Part print with two shaded views. Sizes in mm from the minimum x, y, z corner. A direction names the side the tool comes from. Round coordinates to 2 decimals unless told otherwise and drop trailing zeros. Order: outer loops, then holes, each group sorted by start corner. A loop starts at its lowest first (then second) coordinate and runs counter-clockwise, first axis right, second up. Notation, with made-up numbers: M 65,-23.75 L 122,-23.75 A12 cw 122,-12.75 Z; hole C 12,65 d4. An arc over 180 degrees is marked long. Return JSON: item names as keys, results as strings. Group by question number.
Item 1: Slice it at D-D on x = 10.5. Write the cut outline in (y, z).
Item 2: Which spindle directions (+Z, -Z, +X, -X, +Y, -Y) get a long thin tool onto all of the face, cutting with end or side? Do the marked faces 4, 5 and 6. Say none if no direction does.
Item 3: Pull direction Z, two halves, no side cores. Call the marked faces 1, 2 and 3: pulls with the +Z half, pulls with the -Z half, needs draft (parallel to the pull), parting line crosses it, or undercut.
Item 4: Slice it at A-A on x = 25.5. Give the number of separate pieces and of enclosed holes in the cut face.
Item 5: Probe line 1 along Z through (x, y) = (9, 37); line 2 along Z through (x, y) = (31, 29.5) (1 decimal); line 3 along X through (y, z) = (62, 39.5). List the from-to ranges inside material, lowest first.
Item 6: Pin check, flat tips, straight feed: pin 1 Ø2 at (y, z) = (55.5, 54) entering from +X; pin 2 Ø3 at (x, z) = (6.5, 30) entering from -Y (1 decimal); pin 3 Ø5 at (y, z) = (61.5, 9.5) entering from -X; pin 4 Ø11 at (y, z) = (37.5, 37.5) entering from -X. Stop position of each tip, or through.
Item 7: Slice it at B-B on y = 37.5. Write the cut outline in (x, z).
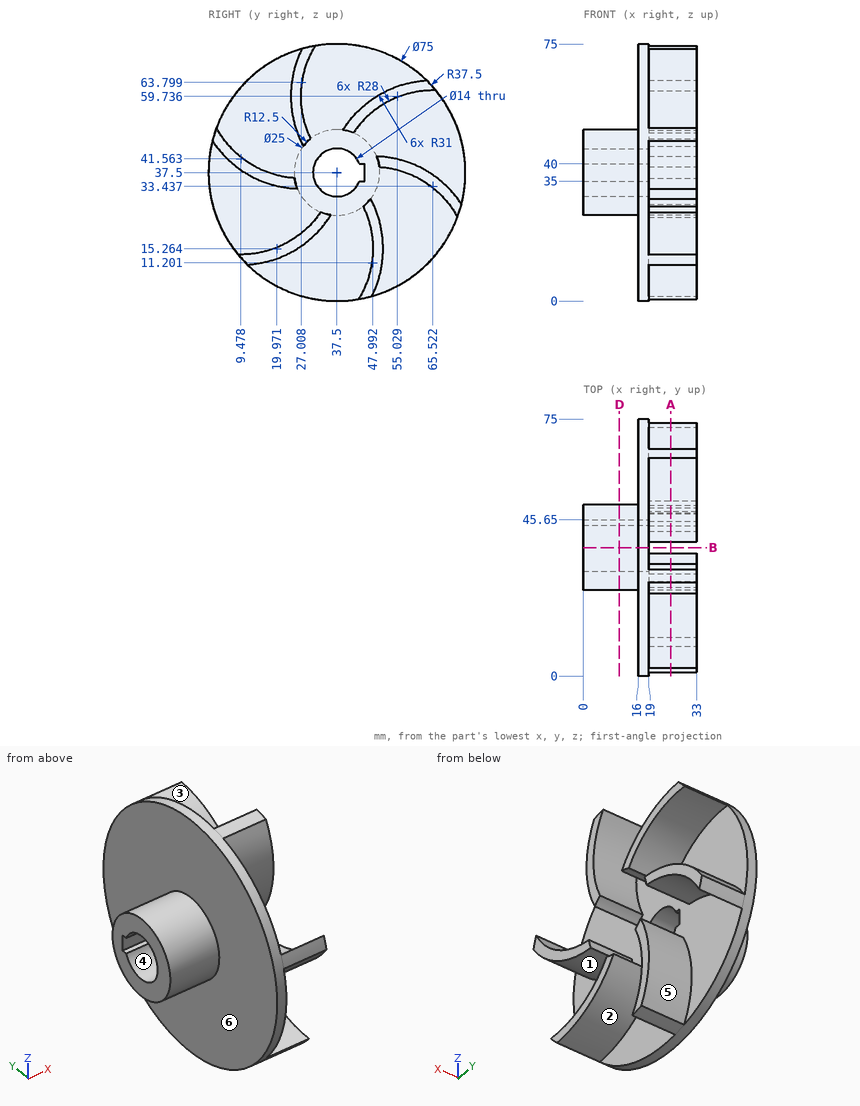
Output values:
{
 "1": {"outline": "C 37.5,37.5 d25; hole M 44.04,35 L 45.65,35 L 45.65,40 L 44.04,40 A7 ccw long Z"},
 "2": {"face 4": "+X, -X", "face 5": "+X", "face 6": "-X"},
 "3": {"face 1": "undercut", "face 2": "pulls with the -Z half", "face 3": "pulls with the +Z half"},
 "4": {"separate pieces": "6", "enclosed holes": "0"},
 "5": {"line 1": "25.01 to 30.52, 44.48 to 49.99", "line 2": "17.9 to 22, 47.1 to 48.2, 71.2 to 74.1", "line 3": "16 to 19"},
 "6": {"pin 1": "x = 19", "pin 2": "y = 26.5", "pin 3": "x = 16", "pin 4": "through"},
 "7": {"outline": "M 0,25 L 16,25 L 16,0 L 19,0 L 19,30.5 L 0,30.5 Z; M 0,44.5 L 19,44.5 L 19,75 L 16,75 L 16,50 L 0,50 Z"}
}
